Geometry check sheet. Reference: drawing and pictorial views, mm from the part's lowest x, y, z. Give positions to 0.01 mm unless a question says otherwise; leave off trailing zeros. Order: outer loops, then holes, each group sorted by start corner. A loop starts at its lowest first (then second) coordinate and runs counter-clockwise, first axis right, second up.
Item 1: Material ranges on line 1 along Y through (x, z) = (1.5, 2.8); line 2 along X through (y, z) = (2.3, 4.4); line 3 along Y through (x, z) = (13.25, 0.8), recorded low to high.
Item 2: Sectioned sample at A-A on z = 2.4. Record the boundary of the cut face in (x, y).
Item 3: Gauge pin test, flat end, axial feed: P1, Ø1, axis at y = 4, z = 4.5, coming from the +X side. Record the tip position at first contact, or that the pin passes through.
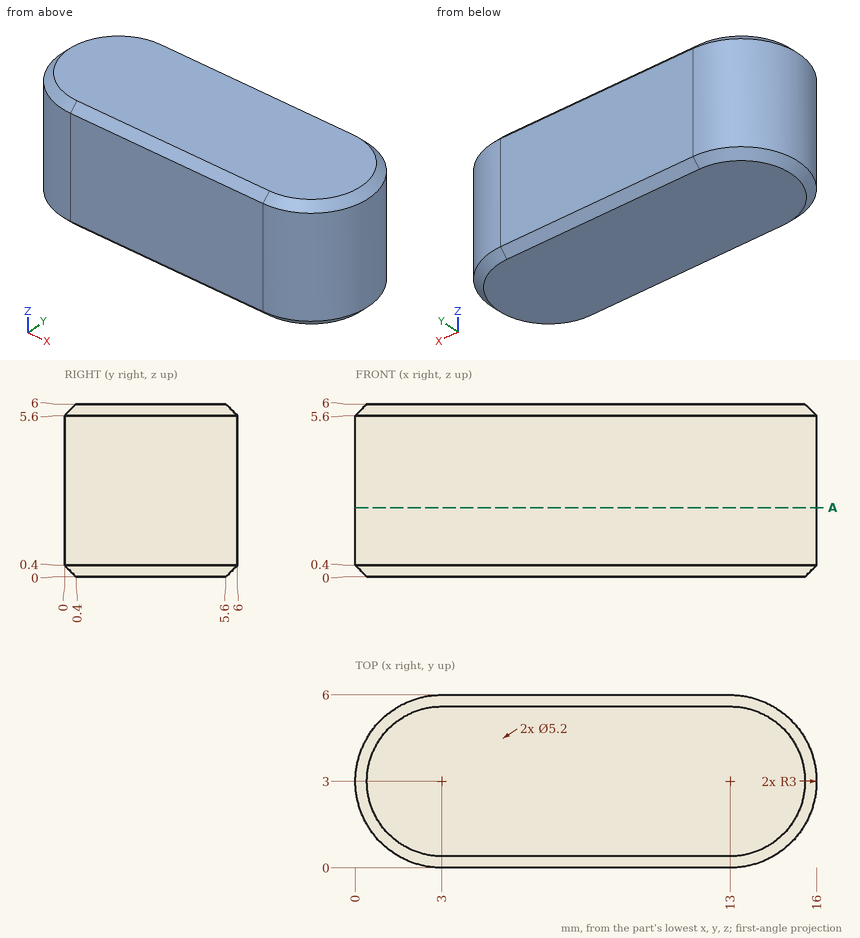
Report:
1. line 1: y = 0.4 to 5.6
1. line 2: x = 0.08 to 15.92
1. line 3: y = 0.01 to 5.99
2. outline: (3, 0) - (13, 0) arc R3 ccw to (13, 6) - (3, 6) arc R3 ccw to start
3. P1: stops at x = 15.96
